Source: three-view drawing plus pictorial views. Frame: mm from the lowest corner of the part. Give positions to 0.01 mm unless a question says otherwise; leave off trailing zeros. Write each loop counter-clockwise with the first axis right and the second up, starting at its lowest first coordinate (ties: lowest second). Pieces come first, ordered by that corner, then holes. Notation, with made-up numbers: M 38.25,9 L 42.25,9 A21 cw 42.25,44 Z; hole C 0,59 d2. An arc over 180 degrees is marked long. One line per question, with ' | ' between items.
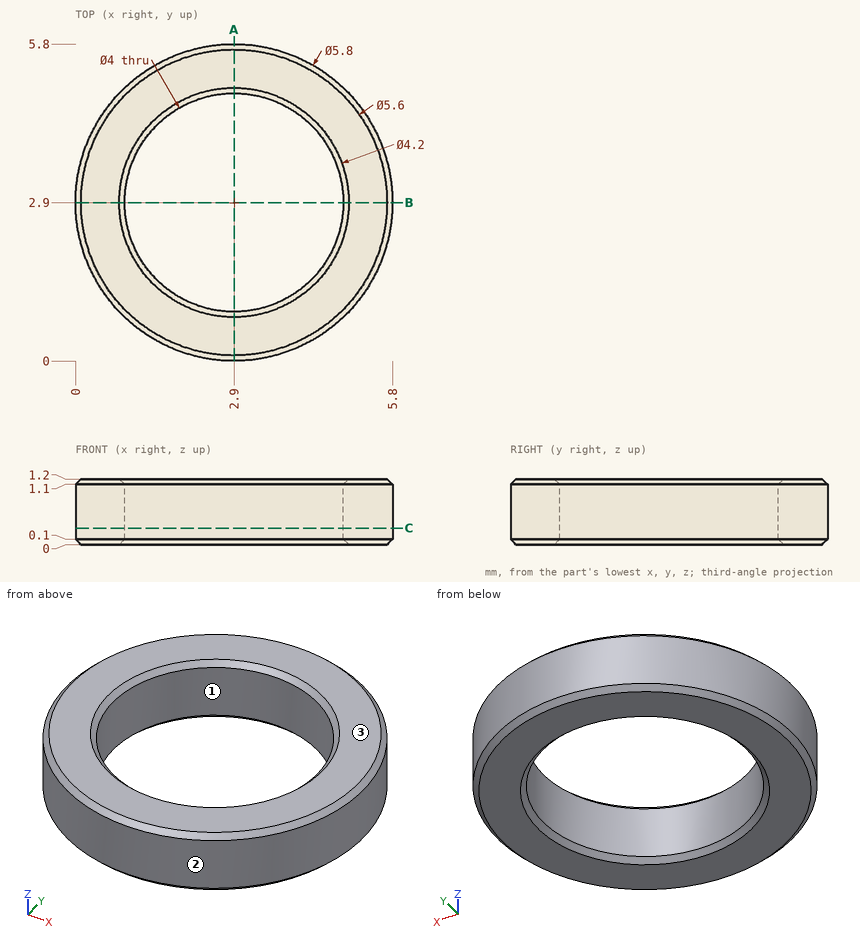
(1) Cut plane A-A, the plane x = 2.9. Return loops of the section in (y, z).
Working result:
outline: M 0,0.1 L 0.1,0 L 0.8,0 L 0.9,0.1 L 0.9,1.1 L 0.8,1.2 L 0.1,1.2 L 0,1.1 Z; M 4.9,0.1 L 5,0 L 5.7,0 L 5.8,0.1 L 5.8,1.1 L 5.7,1.2 L 5,1.2 L 4.9,1.1 Z
(2) Cut plane C-C, the plane z = 0.3. Return loops of the section in (x, y).
Working result:
outline: C 2.9,2.9 d5.8; hole C 2.9,2.9 d4
(3) Material intervals for L1, parallel to Y at x = 2.9, z = 0.85; L2, parallel to Y at x = 3.5, z = 0.25, sorted ascending. Write a range as [from, to].
Working result:
L1: y = [0, 0.9], [4.9, 5.8] | L2: y = [0.06, 0.99], [4.81, 5.74]
(4) Draft query along X for the marked faces 1, 2 and 3. Return one class per face: released by +X, released by -X, zero draft, split by the parting line, or undercut.
Working result:
face 1: undercut | face 2: split by the parting line | face 3: zero draft
